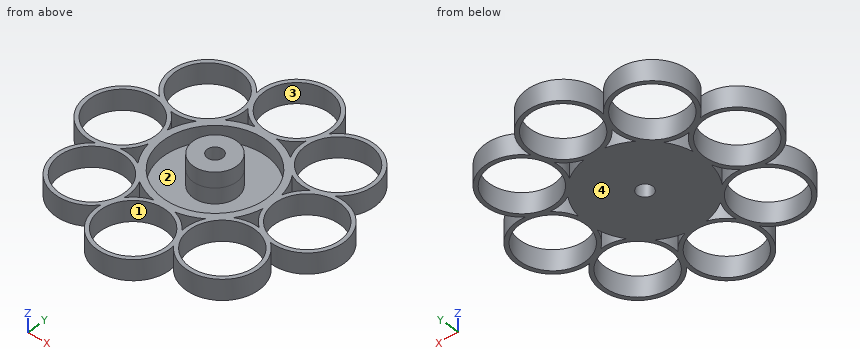
from build123d import *

# Parameters (mm, degrees)
SKETCH1_R           = 3
SKETCH1_R_2         = 12.7
BOSS_EXTRUDE1_DEPTH = 8
SKETCH4_R           = 20
SKETCH4_R_2         = 8.5
CUT_EXTRUDE2_DEPTH  = 6
SKETCH5_R           = 8.5
SKETCH5_R_2         = 3
BOSS_EXTRUDE3_DEPTH = 6


with BuildPart() as part:
    # Sketch1 → Boss-Extrude1 (new body)
    with BuildSketch(Plane.XY):
        with BuildLine():
            ThreePointArc((-14.086428596, 34.007646961), (-35.355339059, 35.355339059), (-34.007646961, 14.086428596))
            ThreePointArc((-34.007646961, 14.086428596), (-50, 0), (-34.007646961, -14.086428596))
            ThreePointArc((-34.007646961, -14.086428596), (-35.355339059, -35.355339059), (-14.086428596, -34.007646961))
            ThreePointArc((-14.086428596, -34.007646961), (0, -50), (14.086428596, -34.007646961))
            ThreePointArc((14.086428596, -34.007646961), (35.355339059, -35.355339059), (34.007646961, -14.086428596))
            ThreePointArc((34.007646961, -14.086428596), (50, 0), (34.007646961, 14.086428596))
            ThreePointArc((34.007646961, 14.086428596), (35.355339059, 35.355339059), (14.086428596, 34.007646961))
            ThreePointArc((14.086428596, 34.007646961), (0, 50), (-14.086428596, 34.007646961))
        make_face()
        Circle(SKETCH1_R, mode=Mode.SUBTRACT)
        with Locations((0, 35.8)):
            Circle(SKETCH1_R_2, mode=Mode.SUBTRACT)
        with Locations((25.314422766, 25.314422766)):
            Circle(SKETCH1_R_2, mode=Mode.SUBTRACT)
        with Locations((35.8, 0)):
            Circle(SKETCH1_R_2, mode=Mode.SUBTRACT)
        with Locations((25.314422766, -25.314422766)):
            Circle(SKETCH1_R_2, mode=Mode.SUBTRACT)
        with Locations((0, -35.8)):
            Circle(SKETCH1_R_2, mode=Mode.SUBTRACT)
        with Locations((-25.314422766, -25.314422766)):
            Circle(SKETCH1_R_2, mode=Mode.SUBTRACT)
        with Locations((-35.8, 0)):
            Circle(SKETCH1_R_2, mode=Mode.SUBTRACT)
        with Locations((-25.314422766, 25.314422766)):
            Circle(SKETCH1_R_2, mode=Mode.SUBTRACT)
        with BuildLine():
            ThreePointArc((-11.227994171, 27.106775805), (-8.03692429, 24.093256305), (-4.078024952, 22.198172458))
            ThreePointArc((-4.078024952, 22.198172458), (-8.637031526, 20.85163865), (-12.812879177, 18.580077372))
            ThreePointArc((-12.812879177, 18.580077372), (-11.353541248, 22.719468579), (-11.227994171, 27.106775805))
        make_face(mode=Mode.SUBTRACT)
        with BuildLine():
            ThreePointArc((11.227994171, 27.106775805), (11.353541248, 22.719468579), (12.812879177, 18.580077372))
            ThreePointArc((12.812879177, 18.580077372), (8.637031526, 20.85163865), (4.078024952, 22.198172458))
            ThreePointArc((4.078024952, 22.198172458), (8.03692429, 24.093256305), (11.227994171, 27.106775805))
        make_face(mode=Mode.SUBTRACT)
        with BuildLine():
            ThreePointArc((27.106775805, 11.227994171), (24.093256305, 8.03692429), (22.198172458, 4.078024952))
            ThreePointArc((22.198172458, 4.078024952), (20.85163865, 8.637031526), (18.580077372, 12.812879177))
            ThreePointArc((18.580077372, 12.812879177), (22.719468579, 11.353541248), (27.106775805, 11.227994171))
        make_face(mode=Mode.SUBTRACT)
        with BuildLine():
            ThreePointArc((27.106775805, -11.227994171), (22.719468579, -11.353541248), (18.580077372, -12.812879177))
            ThreePointArc((18.580077372, -12.812879177), (20.85163865, -8.637031526), (22.198172458, -4.078024952))
            ThreePointArc((22.198172458, -4.078024952), (24.093256305, -8.03692429), (27.106775805, -11.227994171))
        make_face(mode=Mode.SUBTRACT)
        with BuildLine():
            ThreePointArc((11.227994171, -27.106775805), (8.03692429, -24.093256305), (4.078024952, -22.198172458))
            ThreePointArc((4.078024952, -22.198172458), (8.637031526, -20.85163865), (12.812879177, -18.580077372))
            ThreePointArc((12.812879177, -18.580077372), (11.353541248, -22.719468579), (11.227994171, -27.106775805))
        make_face(mode=Mode.SUBTRACT)
        with BuildLine():
            ThreePointArc((-11.227994171, -27.106775805), (-11.353541248, -22.719468579), (-12.812879177, -18.580077372))
            ThreePointArc((-12.812879177, -18.580077372), (-8.637031526, -20.85163865), (-4.078024952, -22.198172458))
            ThreePointArc((-4.078024952, -22.198172458), (-8.03692429, -24.093256305), (-11.227994171, -27.106775805))
        make_face(mode=Mode.SUBTRACT)
        with BuildLine():
            ThreePointArc((-27.106775805, -11.227994171), (-24.093256305, -8.03692429), (-22.198172458, -4.078024952))
            ThreePointArc((-22.198172458, -4.078024952), (-20.85163865, -8.637031526), (-18.580077372, -12.812879177))
            ThreePointArc((-18.580077372, -12.812879177), (-22.719468579, -11.353541248), (-27.106775805, -11.227994171))
        make_face(mode=Mode.SUBTRACT)
        with BuildLine():
            ThreePointArc((-18.580077372, 12.812879177), (-20.85163865, 8.637031526), (-22.198172458, 4.078024952))
            ThreePointArc((-22.198172458, 4.078024952), (-24.093256305, 8.03692429), (-27.106775805, 11.227994171))
            ThreePointArc((-27.106775805, 11.227994171), (-22.719468579, 11.353541248), (-18.580077372, 12.812879177))
        make_face(mode=Mode.SUBTRACT)
    extrude(amount=BOSS_EXTRUDE1_DEPTH)

    # Sketch4 → Cut-Extrude2 (cut)
    with BuildSketch(Plane.XY.offset(8)):
        Circle(SKETCH4_R)
        Circle(SKETCH4_R_2, mode=Mode.SUBTRACT)
    extrude(amount=-CUT_EXTRUDE2_DEPTH, mode=Mode.SUBTRACT)

    # Sketch5 → Boss-Extrude3 (add)
    with BuildSketch(Plane.XY.offset(8)):
        Circle(SKETCH5_R)
        Circle(SKETCH5_R_2, mode=Mode.SUBTRACT)
    extrude(amount=BOSS_EXTRUDE3_DEPTH)


solid = part.part
For this review, take the finished solid that the model builds, in its own axes (mm). Face numbers are marked on the shaded views. A direction names the side the tool comes from. Round coordinates to 2 decimals unless told otherwise and drop trailing zeros. Write each loop counter-clockwise with the first axis right and the second up, starting at its lowest first coordinate (ties: lowest second). Pieces come first, ordered by that corner, then holes. Notation, with made-up numbers: M 24,-29 L 37,-29 A26 ccw 37,1 Z; hole C 71.5,23.5 d1. An arc over 180 degrees is marked long. Write item = value, one per line. Start each with the question number.
(1) For line 1 along Y through (x, z) = (9.5, 3.5); line 2 along X through (y, z) = (34.5, 3); line 3 along X through (y, z) = (24.5, 7.75), list the stretches that pass through material, from the lowest coordinate up.
(2) We need section D-D (z = 11.25). Give the boundary of the cut face in (x, y).
(3) We need section B-B (y = -32). Give the boundary of the cut face in (x, z), then the cut area to 3 significant figures.
(4) The part is to be moulded in two halves that separate along X. For the marked faces 3 and 4, say which applies: +X half, -X half, draft (parallel to the pull), parting line (faces both ways), or undercut.
(5) We need section C-C (x = 35.8). Give the boundary of the cut face in (y, z), then the cut area to 3 significant figures.
(6) We need section A-A (x = -28.5). Give the boundary of the cut face in (y, z), then the cut area to 3 significant figures.
(7) Clearance check with flat-ended pins moving along their axes: pin 1 Ø12 at (x, y) = (6.5, 38) entering from +Z; pin 2 Ø24 at (x, y) = (0, 0) entering from +Z; pin 3 Ø8 at (y, z) = (-30.5, 4.5) entering from -X; pin 4 Ø4 at (x, z) = (4, 8) entering from -Y. State where each tip first meets the part, or that it passes through.
(8) For the marked faces 1 and 2, list the 3-axis set-ups (+Z, -Z, +X, -X, +Y, -Y) from which the entire face can be reached by the end or side of a thin tool; tool diameter is ignored.
Results found:
q1.line_1 = -46.35 to -44.23, -27.37 to -25.25, -20.47 to -17.6, 17.6 to 20.47, 25.25 to 27.37, 44.23 to 46.35
q1.line_2 = -36.14 to -34.08, -16.54 to -14.49, -14.14 to -12.63, 12.63 to 14.14, 14.49 to 16.54, 34.08 to 36.14
q1.line_3 = -39.49 to -37.99, -12.64 to -11.14, -8.6 to -5.8, 5.8 to 8.6, 11.14 to 12.64, 37.99 to 39.49
q2.outline = C 0,0 d17; hole C 0,0 d6
q3.outline = M -37.84,0 L -36.11,0 L -36.11,8 L -37.84,8 Z; M -14.52,0 L -12.12,0 L -12.12,8 L -14.52,8 Z; M 12.12,0 L 14.52,0 L 14.52,8 L 12.12,8 Z; M 36.11,0 L 37.84,0 L 37.84,8 L 36.11,8 Z
q3.area = 66.1 mm²
q4.face_3 = undercut
q4.face_4 = draft
q5.outline = M -34.89,0 L -32.48,0 L -32.48,8 L -34.89,8 Z; M -18.15,0 L -15.74,0 L -15.74,8 L -18.15,8 Z; M -14.2,0 L -12.7,0 L -12.7,8 L -14.2,8 Z; M 12.7,0 L 14.2,0 L 14.2,8 L 12.7,8 Z; M 15.74,0 L 18.15,0 L 18.15,8 L 15.74,8 Z; M 32.48,0 L 34.89,0 L 34.89,8 L 32.48,8 Z
q5.area = 101 mm²
q6.outline = M -39.15,0 L -37.61,0 L -37.61,8 L -39.15,8 Z; M -13.02,0 L -10.39,0 L -10.39,8 L -13.02,8 Z; M 10.39,0 L 13.02,0 L 13.02,8 L 10.39,8 Z; M 37.61,0 L 39.15,0 L 39.15,8 L 37.61,8 Z
q6.area = 66.8 mm²
q7.pin_1 = 8
q7.pin_2 = 14
q7.pin_3 = -39.46
q7.pin_4 = -49.86
q8.face_1 = +Z, -Z
q8.face_2 = +Z
